Geometry check sheet. Reference: the model listing, model coordinates, mm. Face numbers are marked on the shaded views. A direction names the side the tool comes from. Round coordinates to 2 decimals unless told otherwise and drop trailing zeros. Order: outer loops, then holes, each group sorted by start corner. A loop starts at its lowest first (then second) coordinate and runs counter-clockwise, first axis right, second up.
(1) Set-up check for the marked faces 1, 2 and 3: record each of +Z, -Z, +X, -X, +Y, -Y from which the full face is reachable in a straight line by a thin tool's end or side.
(2) Sectioned sample at A-A (z = 4.75). Record the boundary of the cut face in (x, y).
(3) Go/stop test with flat-tipped pins: pin 1 (6 mm diameter, centred on y = -2.5, z = -4, fed in from -X); pin 2 (3 mm diameter, centred on x = 2, z = -2.5, fed in from +Y); pin 3 (1 mm diameter, centred on x = -1.5, y = 0.5, fed in from +Z). Record where each tip stops, or that it passes through.
(4) Material ranges on line 1 along Y through (x, z) = (0, -8); line 2 along Z through (x, y) = (-2.75, 3); line 3 along Y through (x, z) = (0.5, -9), recorded low to high.
(5) Release check for a two-part mould opening along X. For the marked faces 4, 5 and 6 record: +X half, -X half, draft (parallel to the pull), parting line (faces both ways), or undercut.
(6) Sectioned sample at B-B (z = -10.75). Record the boundary of the cut face in (x, y), plus the area to 3 significant figures.
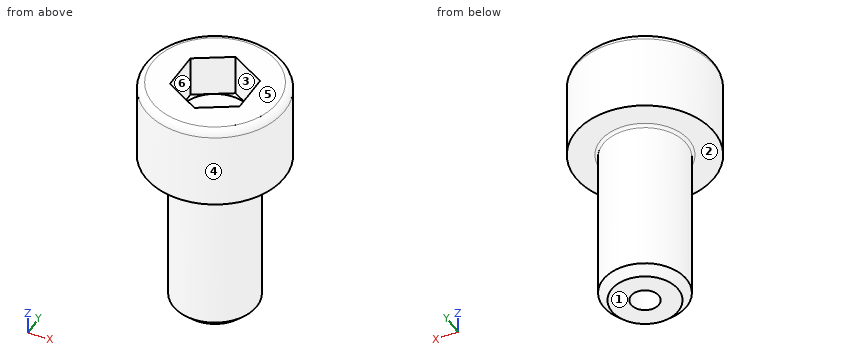
from build123d import *

# Parameters (mm, degrees)
CUT_EXTRUDE1_DEPTH = 3
FILLET1_R          = 0.5
CHAMFER1_SIZE      = 0.6
FILLET2_R          = 0.2


with BuildPart() as part:
    # Sketch3 → Revolve1 (revolve)
    with BuildSketch(Plane(origin=(0, 0, 0), x_dir=(0, 0, -1), z_dir=(1, 0, 0)), mode=Mode.PRIVATE) as revolve1_sk:
        Polygon((-6, 1), (-6, 5), (0, 5), (0, 3), (12, 3), (12, 1), align=None)
    revolve(revolve1_sk.sketch.rotate(Axis((0, 0, 6), (0, 0, -1)), 90), axis=Axis((0, 0, 6), (0, 0, -1)))

    # Sketch4 → Cut-Extrude1 (cut)
    with BuildSketch(Plane.XY.offset(6)):
        Polygon((0, 2.886751346), (-2.5, 1.443375673), (-2.5, -1.443375673), (0, -2.886751346), (2.5, -1.443375673), (2.5, 1.443375673), align=None)
    extrude(amount=-CUT_EXTRUDE1_DEPTH, mode=Mode.SUBTRACT)

    # Fillet1
    fillet1_edges = [part.edges().sort_by_distance(p)[0] for p in [
        (-5, 0, 6),
    ]]
    fillet(fillet1_edges, radius=FILLET1_R)

    # Chamfer1
    chamfer1_edges = [part.edges().sort_by_distance(p)[0] for p in [
        (-3, 0, -12),
    ]]
    chamfer(chamfer1_edges, length=CHAMFER1_SIZE)

    # Cut-Extrude2 cone 1 section (through the dimple's axis) → Cut-Extrude2 (revolve, cut)
    with BuildSketch(Plane(origin=(0, 0, 3), x_dir=(0, -1, 0), z_dir=(1, 0, 0))):
        Polygon((0, 0), (2.5, 0), (0, 1.443375673), align=None)
    revolve(axis=Axis((0, 0, 3), (0, 0, -1)), mode=Mode.SUBTRACT)

    # Fillet2
    fillet2_edges = [part.edges().sort_by_distance(p)[0] for p in [
        (-3, 0, 0),
    ]]
    fillet(fillet2_edges, radius=FILLET2_R)


solid = part.part
Answer below:
1. face 1: -Z, +X, -X, +Y, -Y
1. face 2: -Z
1. face 3: +Z
2. outline: circle Ø10 at (0, 0); hole (-2.5, -1.44) - (0, -2.89) - (2.5, -1.44) - (2.5, 1.44) - (0, 2.89) - (-2.5, 1.44) - close
3. pin 1: stops at x = -3
3. pin 2: stops at y = 2.96
3. pin 3: stops at z = 2.76
4. line 1: y = -3 to -1, 1 to 3
4. line 2: z = 0 to 6
4. line 3: y = -2.96 to -0.87, 0.87 to 2.96
5. face 4: parting line
5. face 5: draft
5. face 6: undercut
6. outline: circle Ø6 at (0, 0); hole circle Ø2 at (0, 0)
6. area: 25.1 mm2
